Part print with two shaded views. Sizes in mm from the minimum x, y, z corner. Give positions to 0.01 mm unless a question says otherwise; leave off trailing zeros. Order: outer loops, then holes, each group sorted by start corner. A loop starts at its lowest first (then second) coordinate and runs counter-clockwise, first axis right, second up. Notation, with made-up numbers: (53, 17.25) - (66, 17.25) arc R35 cw to (66, 56.25) - close; hole circle Ø4 at (21, 68.25). An arc over 180 degrees is marked (long way). Return JSON: item names as keys, results as strings. Group by question number.
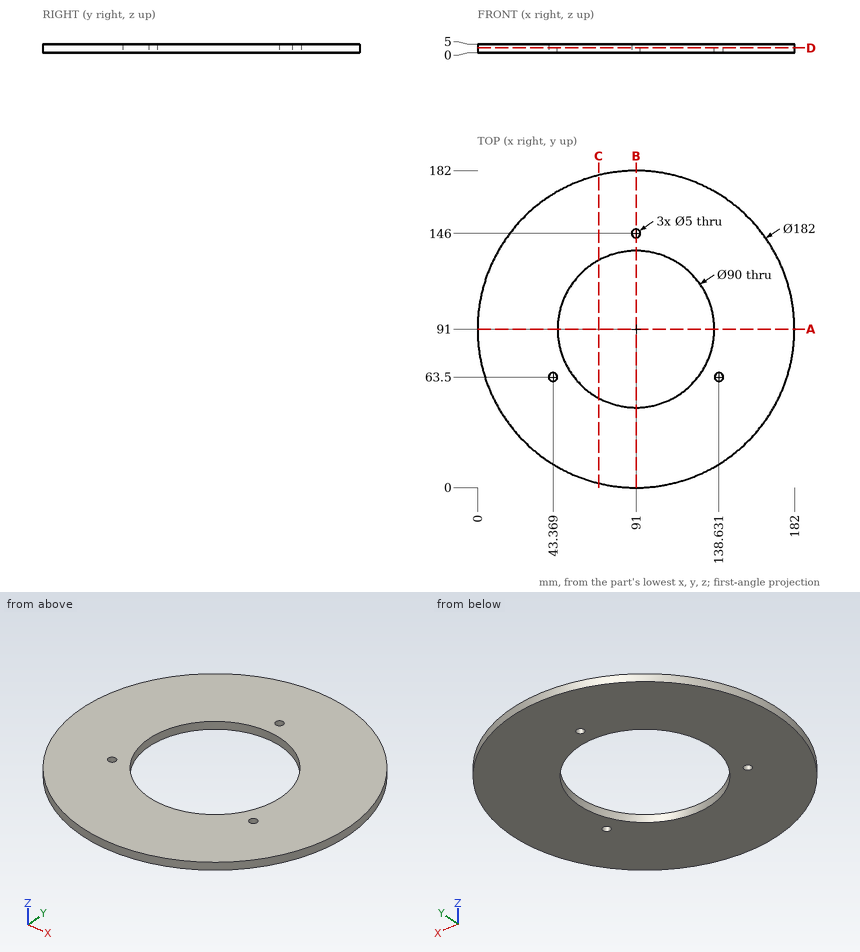
(1) Drill centre lines: L1, parallel to Y at x = 91, z = 3.55; L2, parallel to Y at x = 102, z = 4.05 (1 decimal); L3, parallel to X at y = 114, z = 3.75 (1 decimal). Where is each one in solid material? Low to high.
(2) Slice it at A-A (y = 91). Give the cut face in (x, z), and give its area (3 significant figures).
(3) Slice it at D-D (z = 2.8). Give the cut face in (x, y), and give its area (3 significant figures).
(4) Slice it at B-B (x = 91). Give the cut face in (y, z).
(5) Slice it at C-C (x = 69.5). Give the cut face in (y, z).
(6) Drop flat-ended pins along their axis: pin 1 Ø2 at (y, z) = (40, 3.5) entering from -X; pin 2 Ø3 at (x, z) = (129, 1) entering from +Y; pin 3 Ø2 at (x, z) = (153, 3.5) entering from -Y. Give the stop position or say it passes through.
Result set:
{
 "1": {"L1": "y = 0 to 46, 136 to 143.5, 148.5 to 182", "L2": "y = 0.7 to 47.4, 134.6 to 181.3", "L3": "x = 3 to 52.3, 129.7 to 179"},
 "2": {"outline": "(0, 0) - (46, 0) - (46, 5) - (0, 5) - close; (136, 0) - (182, 0) - (182, 5) - (136, 5) - close", "area": "460 mm²"},
 "3": {"outline": "circle Ø182 at (91, 91); hole circle Ø5 at (43.37, 63.5); hole circle Ø90 at (91, 91); hole circle Ø5 at (91, 146); hole circle Ø5 at (138.63, 63.5)", "area": "19,600 mm²"},
 "4": {"outline": "(0, 0) - (46, 0) - (46, 5) - (0, 5) - close; (136, 0) - (143.5, 0) - (143.5, 5) - (136, 5) - close; (148.5, 0) - (182, 0) - (182, 5) - (148.5, 5) - close"},
 "5": {"outline": "(2.58, 0) - (51.47, 0) - (51.47, 5) - (2.58, 5) - close; (130.53, 0) - (179.42, 0) - (179.42, 5) - (130.53, 5) - close"},
 "6": {"pin 1": "stops at x = 14.97", "pin 2": "stops at y = 174.36", "pin 3": "stops at y = 23.47"}
}
